Part print with two shaded views. Sizes in mm from the minimum x, y, z corner. Coordinates: 2 decimals unless noted, no trailing zeros. Loops run counter-clockwise (first coordinate to the right, second up) from the corner with the lowest first, then second, coordinate; pieces in that order, holes last.
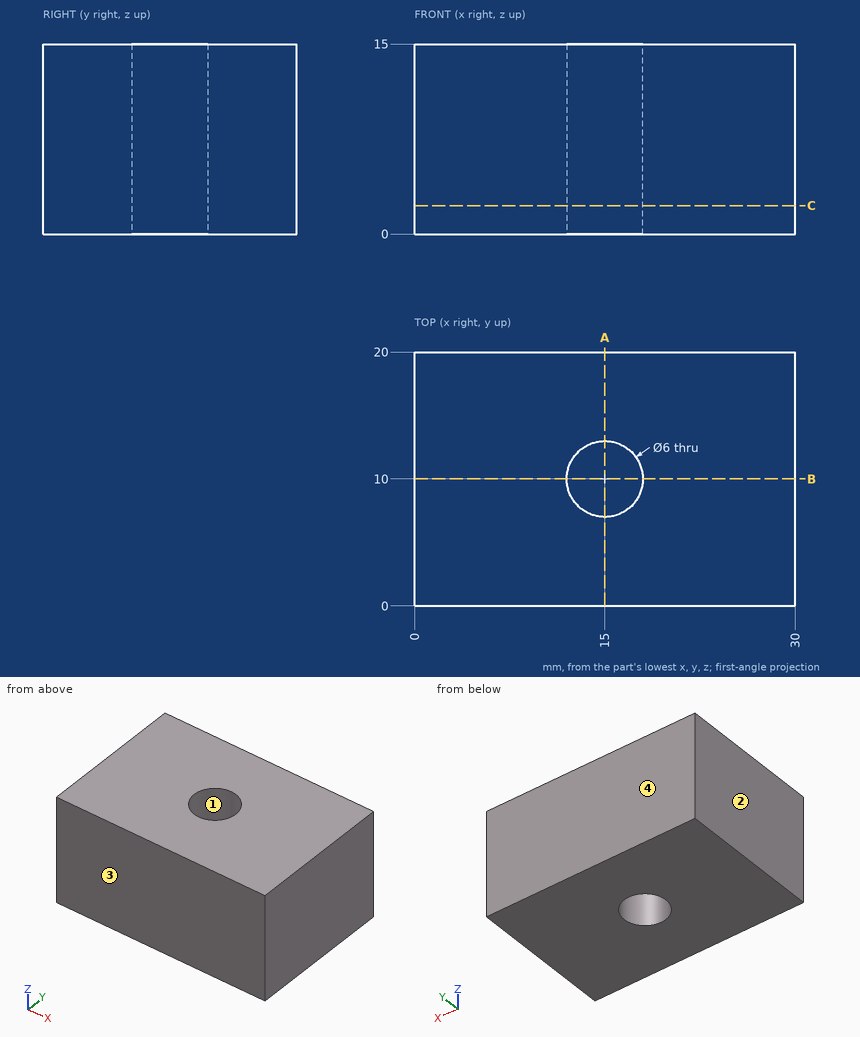
Q1. Slice it at C-C (z = 2.25). List the corners of the cut face in (x, y).
Answers:
outline: (0, 0) - (30, 0) - (30, 20) - (0, 20) - close; hole circle Ø6 at (15, 10)
Q2. Drill centre lines: line 1 (Y direction, x = 15, z = 10.5); line 2 (X direction, y = 10, z = 9); line 3 (Y direction, x = 16.25, z = 4.5). Where is each one in solid material? Low to high.
Answers:
line 1: y = 0 to 7, 13 to 20
line 2: x = 0 to 12, 18 to 30
line 3: y = 0 to 7.27, 12.73 to 20
Q3. Mould opens along Y. For the marked faces 1, 2, 3 and 4 say: +Y half, -Y half, draft (parallel to the pull), parting line (faces both ways), or undercut.
Answers:
face 1: undercut
face 2: draft
face 3: -Y half
face 4: +Y half
Q4. Slice it at A-A (x = 15). List the corners of the cut face in (y, z).
Answers:
outline: (0, 0) - (7, 0) - (7, 15) - (0, 15) - close; (13, 0) - (20, 0) - (20, 15) - (13, 15) - close
Q5. Slice it at B-B (y = 10). List the corners of the cut face in (x, z).
Answers:
outline: (0, 0) - (12, 0) - (12, 15) - (0, 15) - close; (18, 0) - (30, 0) - (30, 15) - (18, 15) - close
